Design review of the part built by this model. Coordinates are the model's own, in mm. Face numbers are marked on the shaded views. A direction names the side the tool comes from. Give positions to 0.01 mm unless a question says otherwise; leave off trailing zeros. Write each loop counter-clockwise with the first axis right and the second up, starting at its lowest first coordinate (ties: lowest second). Pieces come first, ordered by that corner, then holes. Notation, with made-up numbers: (-22, 12.5) -> (22, 12.5) arc R28 cw to (22, 38.5) -> close; hole circle Ø4 at (-22, 17.5). An arc over 180 degrees is marked (long way). Write each question's results on one line, items separated by ' | '. Start each with the question number.
(1) Take a section at B-B (z = 0). State the section outline as (x, y) points.
(2) Clearance check with flat-ended pins moving along their axes: pin 1 (4 mm diameter, centred on x = -29, y = 524, fed in from -Z); pin 2 (4 mm diameter, centred on x = -3.5, y = 521, fed in from +Z); pin 3 (5 mm diameter, centred on y = 527, z = 12.5, fed in from -X). State where each tip first meets the part, or that it passes through.
(3) To check wall thickness, follow probe 1 along X at (y, z) = (527.8, 0); probe 2 along Z at (x, y) = (0, 524.75). State the ranges of each line that lie inside material, in increasing order.
(4) Take a section at C-C (y = 520.25). State the section outline as (x, z) points, plus the area to 3 significant figures.
(5) For the marked faces 4 and 5, list the 3-axis set-ups (+Z, -Z, +X, -X, +Y, -Y) from which the entire face can be reached by the end or side of a thin tool; tool diameter is ignored.
(6) Mouldability with a two-part tool opening along Z and no side actions: class the marked faces 1, 2 and 3 as released by +Z, released by -Z, zero draft, split by the parting line, or undercut.
(7) Take a section at D-D (y = 530.5). State the section outline as (x, z) points, plus the area to 3 significant figures.
(8) Take a section at A-A (x = 0). State the section outline as (y, z) points.
from build123d import *


with BuildPart() as part:
    # Sketch1 → Revolve1 (revolve)
    with BuildSketch(Plane.XY):
        Polygon((15, 517), (35, 517), (40, 522), (40, 529), (35, 529), (35, 526), (25, 526), (25, 532), (15, 532), align=None)
    revolve(axis=Axis((0, 517, 0), (0, 1, 0)))


solid = part.part
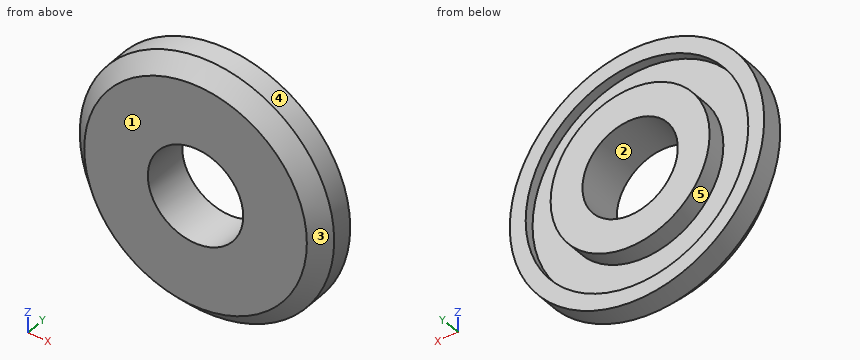
Report:
1) outline: (-40, 522) -> (-35, 517) -> (-15, 517) -> (-15, 532) -> (-25, 532) -> (-25, 526) -> (-35, 526) -> (-35, 529) -> (-40, 529) -> close; (15, 517) -> (35, 517) -> (40, 522) -> (40, 529) -> (35, 529) -> (35, 526) -> (25, 526) -> (25, 532) -> (15, 532) -> close
2) pin 1: z = -29.51 | pin 2: z = 39.96 | pin 3: x = -38.73
3) probe 1: -40 to -35, -25 to -15, 15 to 25, 35 to 40 | probe 2: -40 to -15, 15 to 40
4) outline: circle Ø76.5 at (0, 0); hole circle Ø30 at (0, 0) | area: 3,890 mm2
5) face 4: +Y, -Y | face 5: +Y
6) face 1: zero draft | face 2: undercut | face 3: split by the parting line
7) outline: circle Ø50 at (0, 0); hole circle Ø30 at (0, 0) | area: 1,260 mm2
8) outline: (517, -35) -> (522, -40) -> (529, -40) -> (529, -35) -> (526, -35) -> (526, -25) -> (532, -25) -> (532, -15) -> (517, -15) -> close; (517, 15) -> (532, 15) -> (532, 25) -> (526, 25) -> (526, 35) -> (529, 35) -> (529, 40) -> (522, 40) -> (517, 35) -> close
